Here's how the part is built. I have some questions about the finished solid (model axes, mm). A direction names the side the tool comes from. Give positions to 0.01 mm unless a question says otherwise; leave off trailing zeros. Order: outer loops, then holes, each group sorted by start corner. A loop starts at its lowest first (then second) coordinate and runs counter-clockwise, first axis right, second up. Notation, with made-up numbers: (-37.75, 62) - (20.25, 62) arc R33 cw to (20.25, 100) - close; hole circle Ø7 at (89, 28.25). An arc over 180 degrees is marked (long way). One line per question, with ' | ' between items.
from build123d import *

# Parameters (mm, degrees)
SKETCH3_R           = 4
BOSS_EXTRUDE2_DEPTH = 14
SKETCH4_R           = 4
BOSS_EXTRUDE3_DEPTH = 10
SKETCH5_R           = 5
BOSS_EXTRUDE4_DEPTH = 2
CUT_EXTRUDE1_DEPTH  = 1.8
SKETCH7_R           = 4
BOSS_EXTRUDE5_DEPTH = 42
SKETCH8_R           = 4
BOSS_EXTRUDE7_DEPTH = 150
SKETCH9_R           = 4
BOSS_EXTRUDE8_DEPTH = 198
SKETCH10_R          = 4
BOSS_EXTRUDE9_DEPTH = 33.1
CUT_EXTRUDE2_DEPTH  = 1.8


with BuildPart() as part:
    # Sketch3 → Boss-Extrude2 (new body)
    with BuildSketch(Plane.XY):
        Circle(SKETCH3_R)
    extrude(amount=BOSS_EXTRUDE2_DEPTH)

    # Sketch4 → Boss-Extrude3 (add)
    with BuildSketch(Plane.XY.offset(14)):
        Circle(SKETCH4_R)
    extrude(amount=BOSS_EXTRUDE3_DEPTH)

    # Sketch5 → Boss-Extrude4 (add)
    with BuildSketch(Plane.XY.offset(24)):
        Circle(SKETCH5_R)
    extrude(amount=BOSS_EXTRUDE4_DEPTH)

    # Sketch6 → Cut-Extrude1 (cut)
    with BuildSketch(Plane(origin=(0, 4, 0), x_dir=(1, 0, 0), z_dir=(0, 1, 0))):
        with BuildLine():
            Line((1.5, -5.5), (1.5, -10.5))
            ThreePointArc((1.5, -10.5), (0, -12), (-1.5, -10.5))
            Line((-1.5, -10.5), (-1.5, -5.5))
            ThreePointArc((-1.5, -5.5), (0, -4), (1.5, -5.5))
        make_face()
    extrude(amount=-CUT_EXTRUDE1_DEPTH, mode=Mode.SUBTRACT)

    # Sketch7 → Boss-Extrude5 (add)
    with BuildSketch(Plane.XY.offset(26)):
        Circle(SKETCH7_R)
    extrude(amount=BOSS_EXTRUDE5_DEPTH)

    # Sketch8 → Boss-Extrude7 (add)
    with BuildSketch(Plane.XY.offset(68)):
        Circle(SKETCH8_R)
    extrude(amount=BOSS_EXTRUDE7_DEPTH)

    # Sketch9 → Boss-Extrude8 (add)
    with BuildSketch(Plane.XY.offset(218)):
        Circle(SKETCH9_R)
    extrude(amount=BOSS_EXTRUDE8_DEPTH)

    # Sketch10 → Boss-Extrude9 (add)
    with BuildSketch(Plane.XY.offset(416)):
        Circle(SKETCH10_R)
    extrude(amount=BOSS_EXTRUDE9_DEPTH)

    # Sketch13 → Cut-Extrude2 (cut)
    with BuildSketch(Plane(origin=(0, 4, 0), x_dir=(1, 0, 0), z_dir=(0, 1, 0))):
        with BuildLine():
            Line((1.5, -440.6), (1.5, -445.6))
            ThreePointArc((1.5, -445.6), (0, -447.1), (-1.5, -445.6))
            Line((-1.5, -445.6), (-1.5, -440.6))
            ThreePointArc((-1.5, -440.6), (0, -439.1), (1.5, -440.6))
        make_face()
    extrude(amount=-CUT_EXTRUDE2_DEPTH, mode=Mode.SUBTRACT)


solid = part.part
1) I'm going to push flat-ended pins straight in: P1, Ø1.5, axis at x = -1, z = 304, coming from the +Y side; P2, Ø0.5, axis at y = 3, z = 7.5, coming from the +X side; P3, Ø0.8, axis at y = 2.5, z = 443.5, coming from the -X side. Where does each tip first touch, or does it pass through?
Model answer:
P1: stops at y = 3.99 | P2: stops at x = 2.9 | P3: stops at x = -3.4
2) I want a section at A-A (y = 0). List the corners of the cut face in (x, z) for me, plus the area to 3 significant figures.
Model answer:
outline: (-5, 24) - (-4, 24) - (-4, 0) - (4, 0) - (4, 24) - (5, 24) - (5, 26) - (4, 26) - (4, 449.1) - (-4, 449.1) - (-4, 26) - (-5, 26) - close | area: 3,600 mm2
3) I want a section at B-B (x = 0). List the corners of the cut face in (y, z) for me.
Model answer:
outline: (-5, 24) - (-4, 24) - (-4, 0) - (4, 0) - (4, 4) - (2.2, 4) - (2.2, 12) - (4, 12) - (4, 24) - (5, 24) - (5, 26) - (4, 26) - (4, 439.1) - (2.2, 439.1) - (2.2, 447.1) - (4, 447.1) - (4, 449.1) - (-4, 449.1) - (-4, 26) - (-5, 26) - close
4) Please list where these lines run through material, in increasing order: L1, parallel to Z at x = 0.25, y = 2.75; L2, parallel to Y at x = -0.75, z = 165; L3, parallel to Z at x = -2.5, y = 3.25.
Model answer:
L1: z = 0 to 4.02, 11.98 to 439.12, 447.08 to 449.1 | L2: y = -3.93 to 3.93 | L3: z = 24 to 26
5) I want a section at C-C (z = 356). List the corners of the cut face in (x, y) for me.
Model answer:
outline: circle Ø8 at (0, 0)
6) On a 3-axis mill with a long thin cutter (end or side, diameter ignored), from which of +Z, -Z, +X, -X, +Y, -Y can I reach the whole of each face in a straight line? I mean faces 1 (the face through (-0.867, -3.905, 234.588)), 2 (the face through (0, 0, 449.1)), 3 (the face through (-0.867, -3.905, 11.832)). Say none if no direction works.
Model answer:
face 1: +Z | face 2: +Z, +X, -X, +Y, -Y | face 3: -Z
